Verification items for the finished model (mm, model axes). A direction names the side the tool comes from. Coordinates: 2 decimals unless noted, no trailing zeros. Order: outer loops, then holes, each group sorted by start corner. A loop starts at its lowest first (then second) coordinate and runs counter-clockwise, first axis right, second up.
Q1. Depth check by flat-ended pin: P1, Ø6, axis at x = 18.5, y = 32.5, coming from the -Z side; P2, Ø1.5, axis at y = 24, z = -9.5, coming from the -X side; P3, Ø4, axis at y = 42, z = -11.5, coming from the -X side. Enter the tip coordinate at first touch or a pass-through.
Q2. Draft check along X on faces 1 (the flat face through (40, 53, -10)), 2 (the flat face through (-13, 0, -10)), 3 (the cylindrical face through (-3.47, 10.14, 15.62)). Enter one of: pulls with the +X half, pulls with the -X half, needs draft (parallel to the pull), parting line crosses it, or undercut.
Q3. Cross-section at D-D, the plane z = 9. Record the boundary of the cut face in (x, y).
Q4. Set-up check for faces 4 (the cylindrical face through (8.767, 10.14, 16.856)), 5 (the cylindrical face through (30.14, 44.119, 18.548)): record each of +Z, -Z, +X, -X, +Y, -Y from which the full face is reachable in a straight line by a thin tool's end or side.
Q5. Thickness scan on line 1 (Y direction, x = 34, z = 0); line 2 (Z direction, x = 11.5, y = 37.5); line 3 (X direction, y = 7.75, z = 0). Record the ranges inside material, lowest first.
Q6. Cross-section at A-A, the plane z = 0. Record the boundary of the cut face in (x, y).
Q7. Cross-section at C-C, the plane z = 17. Record the boundary of the cut face in (x, y).
Q8. Cross-section at B-B, the plane y = 6. Record the boundary of the cut face in (x, z).
from build123d import *

# Parameters (mm, degrees)
SKETCH_2_R   = 19
SKETCH_2_R_2 = 16


with BuildPart() as part:
    # 扫描1: sweep along a path in 草图1
    with BuildLine(Plane.XY) as sweep_1_path:
        Line((0, 0), (0, 20))
        ThreePointArc((0, 20), (5.857864376, 34.142135624), (20, 40))
        Line((20, 40), (40, 40))
    # 草图2 → 扫描1 (sweep)
    with BuildSketch(Plane(origin=(0, 0, 0), x_dir=(1, 0, 0), z_dir=(0, 1, 0))):
        Circle(SKETCH_2_R)
        Circle(SKETCH_2_R_2, mode=Mode.SUBTRACT)
    sweep(path=sweep_1_path.line)


solid = part.part
Check values:
1. P1: stops at z = -18.48
1. P2: stops at x = -16.66
1. P3: stops at x = -9.66
2. face 1: pulls with the +X half
2. face 2: needs draft
2. face 3: undercut
3. outline: (-16.73, 0) - (-13.23, 0) - (-13.23, 20) arc R33.23 cw to (20, 53.23) - (40, 53.23) - (40, 56.73) - (20, 56.73) arc R36.73 ccw to (-16.73, 20) - close; (13.23, 0) - (16.73, 0) - (16.73, 20) arc R3.27 cw to (20, 23.27) - (40, 23.27) - (40, 26.77) - (20, 26.77) arc R6.77 ccw to (13.23, 20) - close
4. face 4: -Y
4. face 5: +X
5. line 1: y = 21 to 24, 56 to 59
5. line 2: z = -18.99 to -15.99, 15.99 to 18.99
5. line 3: x = -19 to -16, 16 to 19
6. outline: (-19, 0) - (-16, 0) - (-16, 20) arc R36 cw to (20, 56) - (40, 56) - (40, 59) - (20, 59) arc R39 ccw to (-19, 20) - close; (16, 0) - (19, 0) - (19, 20) arc R1 cw to (20, 21) - (40, 21) - (40, 24) - (20, 24) arc R4 ccw to (16, 20) - close
7. outline: (-8.49, 0) - (8.49, 0) - (8.49, 20) arc R11.51 cw to (20, 31.51) - (40, 31.51) - (40, 48.49) - (20, 48.49) arc R28.49 ccw to (-8.49, 20) - close
8. outline: circle Ø38 at (0, 0); hole circle Ø32 at (0, 0)
